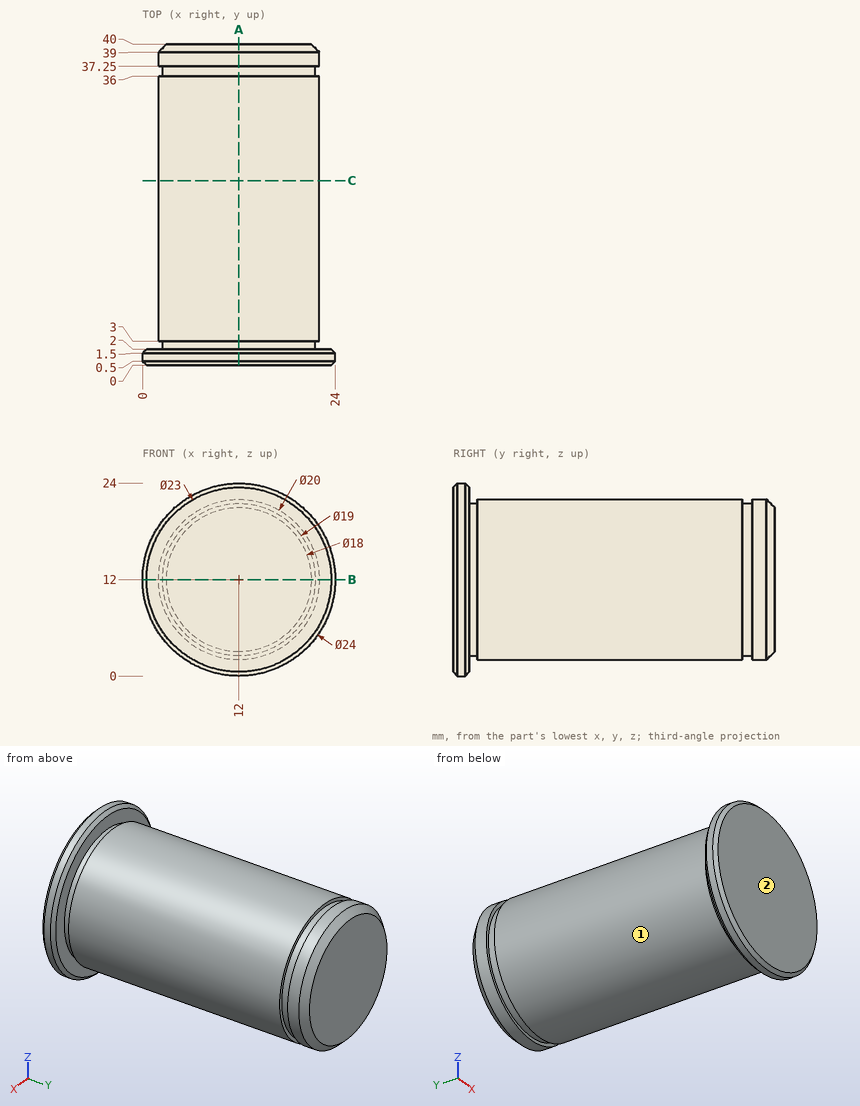
Study the drawing (mm; zero at the part's minimum x, y, z) and answer. A direction names the side the tool comes from. Coordinates: 2 decimals unless noted, no trailing zeros. Loops run counter-clockwise (first coordinate to the right, second up) from the corner with the lowest first, then second, coordinate; pieces in that order, holes last. Notation, with made-up numbers: M 32,48 L 67,48 A27 cw 67,76 Z; hole C 6.25,53.25 d7. An arc over 180 degrees is marked long. Answer in a Markdown table with one row per item.
1) Find section B-B (z = 12). Determine the outline of the cut face in (x, y), then the cut area to 3 significant figures.
Answers below:
| item | result |
|---|---|
| outline | M 0,0.5 L 0.5,0 L 23.5,0 L 24,0.5 L 24,1.5 L 23.5,2 L 21.5,2 L 21.5,3 L 22,3 L 22,36 L 21.5,36 L 21.5,37.25 L 22,37.25 L 22,39 L 21,40 L 3,40 L 2,39 L 2,37.25 L 2.5,37.25 L 2.5,36 L 2,36 L 2,3 L 2.5,3 L 2.5,2 L 0.5,2 L 0,1.5 Z |
| area | 804 mm^2 |
2) Given pin 1 (2 mm diameter, centred on x = 18, z = 7, fed in from -Y); pin 2 (6 mm diameter, centred on x = 12.5, y = 17.5, fed in from -Z); pin 3 (2 mm diameter, centred on x = 8.5, y = 5.5, fed in from -Z); pin 4 (4 mm diameter, centred on x = 18, y = 12, fed in from -Z), each flat-ended and moving along its own axis, determine where each tip first touches the part or whether it passes through.
Answers below:
| item | result |
|---|---|
| pin 1 | y = 0 |
| pin 2 | z = 2 |
| pin 3 | z = 2.32 |
| pin 4 | z = 2.83 |
3) Find section A-A (x = 12). Determine the outline of the cut face in (y, z), then the cut area to 3 significant figures.
Answers below:
| item | result |
|---|---|
| outline | M 0,0.5 L 0.5,0 L 1.5,0 L 2,0.5 L 2,2.5 L 3,2.5 L 3,2 L 36,2 L 36,2.5 L 37.25,2.5 L 37.25,2 L 39,2 L 40,3 L 40,21 L 39,22 L 37.25,22 L 37.25,21.5 L 36,21.5 L 36,22 L 3,22 L 3,21.5 L 2,21.5 L 2,23.5 L 1.5,24 L 0.5,24 L 0,23.5 Z |
| area | 804 mm^2 |
4) Find section C-C (y = 23). Determine the outline of the cut face in (x, z).
Answers below:
| item | result |
|---|---|
| outline | C 12,12 d20 |
5) Find the intervals of material crossed by probe 1 along Y at (x, z) = (20.25, 6.5); probe 2 along Y at (x, z) = (2.75, 17); probe 3 along Z at (x, y) = (11, 18.5), in increasing order.
Answers below:
| item | result |
|---|---|
| probe 1 | 0 to 2, 3 to 36, 37.25 to 39.08 |
| probe 2 | 0 to 2 |
| probe 3 | 2.05 to 21.95 |
6) Which of the six approach directions +Z, -Z, +X, -X, +Y, -Y give full straight-line access (tool end or side, diameter ignored) to the marked faces 1 and 2?
Answers below:
| item | result |
|---|---|
| face 1 | +Y |
| face 2 | +Z, -Z, +X, -X, -Y |
